Work out the finished part from the listing and answer in its coordinate system (mm). A direction names the side the tool comes from. Coordinates: 2 decimals unless noted, no trailing zeros. Order: outer loops, then holes, each group sorted by start corner. A loop starts at its lowest first (then second) coordinate and runs counter-clockwise, first axis right, second up.
1. Find the intervals of material crossed by probe 1 along Y at (x, z) = (-44.7, 6.5); probe 2 along Y at (x, z) = (-140, 3.75); probe 3 along X at (y, z) = (-165.5, 7), in increasing order.
2. The part is cut by section D-D, the plane y = 163. Give the vertices of the cut face in (x, z), then the cut area to 3 significant figures.
3. A tool of negligible diameter and unlimited length cuts with its end or side. For faces 4 (the flat face through (-65, 3, 0)), 5 (the cylindrical face through (217, -15, 8)), from which of +Z, -Z, +X, -X, +Y, -Y can it reach the whole face along a straight path? Write none if from no direction.
4. Determine the mould class of faces 1 (the cylindrical face through (-227.35, 159.74, 7.6)), 2 (the flat face through (-275, -3, 7)), 3 (the flat face through (163.46, -130.91, 7.6)) for opening direction X: +X half, -X half, draft (parallel to the pull), parting line (faces both ways), or undercut.
5. The part is cut by section A-A, the plane x = -235.2. Give the vertices of the cut face in (y, z).
6. The part is cut by section B-B, the plane z = 11.5. Give the vertices of the cut face in (x, y), then the cut area to 3 significant figures.
7. The part is cut by section C-C, the plane x = 217. Give the vertices of the cut face in (y, z).
8. Flat-ended cylindrical pins translate along their axes: pin 1 Ø11.5 at (x, y) = (-140, -163) entering from -Z; pin 2 Ø19.5 at (x, y) = (-235.2, 163) entering from +Z; pin 3 Ø3 at (x, z) = (67, 11) entering from +Y; pin 4 Ø1 at (x, z) = (58, 11.5) entering from +Y. Find the tip coordinate at first contact, or state that the pin passes through.
```python
from build123d import *

# Parameters (mm, degrees)
SKETCH_1_W          = 550
SKETCH_1_H          = 390
EXTRUDE_1_DEPTH     = 15
SKETCH_2_R          = 8.5
SKETCH_2_R_2        = 6.5
CUT_EXTRUDE_1_DEPTH = 15


with BuildPart() as part:
    # 草图1 → 凸台-拉伸1 (new body)
    with BuildSketch(Plane.XY):
        Rectangle(SKETCH_1_W, SKETCH_1_H)
    extrude(amount=EXTRUDE_1_DEPTH)

    # 草图2 → 切除-拉伸1 (cut)
    with BuildSketch(Plane.XY.offset(15)):
        with Locations((-235.2, 163)):
            Circle(SKETCH_2_R)
        with Locations((-235.2, -163)):
            Circle(SKETCH_2_R)
        with Locations((-140, -163)):
            Circle(SKETCH_2_R_2)
        with Locations((-44.7, -163)):
            Circle(SKETCH_2_R)
        with Locations((-140, 163)):
            Circle(SKETCH_2_R_2)
        with Locations((-44.7, 163)):
            Circle(SKETCH_2_R)
        Polygon((55, 195), (275, 65), (275, 195), align=None)
        Polygon((55, -195), (275, -65), (275, -195), align=None)
        with BuildLine():
            Line((228, 4), (228, -4))
            ThreePointArc((228, -4), (217, -15), (206, -4))
            Line((206, -4), (206, 4))
            ThreePointArc((206, 4), (217, 15), (228, 4))
        make_face()
    extrude(amount=-CUT_EXTRUDE_1_DEPTH, mode=Mode.SUBTRACT)


solid = part.part
```
Geometry says:
1. probe 1: y = -195 to -171.5, -154.5 to 154.5, 171.5 to 195
1. probe 2: y = -195 to -169.5, -156.5 to 156.5, 169.5 to 195
1. probe 3: x = -275 to -243.32, -227.08 to -146, -134 to -52.82, -36.58 to 104.92
2. outline: (-275, 0) - (-243.7, 0) - (-243.7, 15) - (-275, 15) - close; (-226.7, 0) - (-146.5, 0) - (-146.5, 15) - (-226.7, 15) - close; (-133.5, 0) - (-53.2, 0) - (-53.2, 15) - (-133.5, 15) - close; (-36.2, 0) - (109.15, 0) - (109.15, 15) - (-36.2, 15) - close
2. area: 5,060 mm2
3. face 4: -Z, +X, -X, +Y, -Y
3. face 5: +Z, -Z
4. face 1: undercut
4. face 2: -X half
4. face 3: +X half
5. outline: (-195, 0) - (-171.5, 0) - (-171.5, 15) - (-195, 15) - close; (-154.5, 0) - (154.5, 0) - (154.5, 15) - (-154.5, 15) - close; (171.5, 0) - (195, 0) - (195, 15) - (171.5, 15) - close
6. outline: (-275, -195) - (55, -195) - (275, -65) - (275, 65) - (55, 195) - (-275, 195) - close; hole circle Ø17 at (-235.2, -163); hole circle Ø17 at (-235.2, 163); hole circle Ø13 at (-140, -163); hole circle Ø13 at (-140, 163); hole circle Ø17 at (-44.7, -163); hole circle Ø17 at (-44.7, 163); hole (206, -4) arc R11 ccw to (228, -4) - (228, 4) arc R11 ccw to (206, 4) - close
6. area: 184,000 mm2
7. outline: (-99.27, 0) - (-15, 0) - (-15, 15) - (-99.27, 15) - close; (15, 0) - (99.27, 0) - (99.27, 15) - (15, 15) - close
8. pin 1: passes through
8. pin 2: stops at z = 15
8. pin 3: stops at y = 188.8
8. pin 4: stops at y = 193.52
